Build history of the part. All positions in model axes, mm. A direction names the side the tool comes from. Round coordinates to 2 decimals unless told otherwise and drop trailing zeros. Order: outer loops, then holes, each group sorted by start corner. A loop starts at its lowest first (then second) coordinate and runs counter-clockwise, first axis right, second up. Notation, with made-up numbers: M 20.25,85.25 L 29.25,85.25 A23 ccw 29.25,98.25 Z; hole C 39,87 d6. An arc over 180 degrees is marked long. Use CSV: the item, a comma, the result in double quotes.
from build123d import *

# Parameters (mm, degrees)
BRACKET_BODY_DEPTH           = 12
RECTANGULAR_WINDOW_CUT_DEPTH = 5
KEYHOLE_SLOT_CUT_DEPTH       = 10
EDGE_NOTCH_CUT_DEPTH         = 2


with BuildPart() as part:
    # Bracket Profile Sketch → Bracket Body (new, symmetric)
    with BuildSketch(Plane.XY):
        with BuildLine():
            Line((2, 0), (18.5, 0))
            ThreePointArc((18.5, 0), (19.75, -1.25), (18.5, -2.5))
            Line((18.5, -2.5), (17, -2.5))
            Line((17, -2.5), (17, -1.268700577))
            Line((17, -1.268700577), (18.441553142, -1.268700577))
            ThreePointArc((18.441553142, -1.268700577), (18.497202853, -1.134350288), (18.441553142, -1))
            Line((18.441553142, -1), (3.021384942, -1))
            ThreePointArc((3.021384942, -1), (1.592049942, -1.592049942), (1, -3.021384942))
            Line((1, -3.021384942), (1, -29))
            Line((1, -29), (0, -29))
            Line((0, -29), (0, -2))
            ThreePointArc((0, -2), (0.585786438, -0.585786438), (2, 0))
        make_face()
    extrude(amount=BRACKET_BODY_DEPTH, both=True)

    # Rectangular Window Sketch → Rectangular Window Cut (cut, symmetric)
    with BuildSketch(Plane.XZ.offset(1)):
        with BuildLine():
            Line((8, -6), (14, -6))
            ThreePointArc((14, -6), (15.414213562, -5.414213562), (16, -4))
            Line((16, -4), (16, 4))
            ThreePointArc((16, 4), (15.414213562, 5.414213562), (14, 6))
            Line((14, 6), (8, 6))
            ThreePointArc((8, 6), (6.585786438, 5.414213562), (6, 4))
            Line((6, 4), (6, -4))
            ThreePointArc((6, -4), (6.585786438, -5.414213562), (8, -6))
        make_face()
    extrude(amount=RECTANGULAR_WINDOW_CUT_DEPTH, both=True, mode=Mode.SUBTRACT)

    # Keyhole Slot Sketch → Keyhole Slot Cut (cut)
    with BuildSketch(Plane(origin=(1, 0, 0), x_dir=(0, 0, -1), z_dir=(1, 0, 0))):
        with BuildLine():
            ThreePointArc((7.546363234, -23.655635881), (4.623576141, -27.52859431), (-3.9e-08, -29))
            Line((-3.9e-08, -29), (12, -29))
            Line((12, -29), (12, -11))
            Line((12, -11), (7.546363234, -23.655635881))
        make_face()
        with BuildLine():
            Line((-7.546363234, -23.655635881), (-12, -11))
            Line((-12, -11), (-12, -29))
            Line((-12, -29), (-3.9e-08, -29))
            ThreePointArc((-3.9e-08, -29), (-4.623576172, -27.528594288), (-7.546363234, -23.655635881))
        make_face()
    extrude(amount=-KEYHOLE_SLOT_CUT_DEPTH, mode=Mode.SUBTRACT)

    # Edge Notch Sketch → Edge Notch Cut (cut)
    with BuildSketch(Plane(origin=(1, 0, 0), x_dir=(0, 0, -1), z_dir=(1, 0, 0))):
        with BuildLine():
            Line((-2.38, -15.84), (-2.38, -18.339079107))
            ThreePointArc((-2.38, -18.339079107), (0, -24.57), (2.38, -18.339079107))
            Line((2.38, -18.339079107), (2.38, -15.84))
            ThreePointArc((2.38, -15.84), (0, -13.46), (-2.38, -15.84))
        make_face()
    extrude(amount=-EDGE_NOTCH_CUT_DEPTH, mode=Mode.SUBTRACT)


solid = part.part
(1) Wall check: line 1 (Y direction, x = 18, z = 5.5); line 2 (X direction, y = -9.75, z = 7.75); line 3 (Y direction, x = 6.5, z = 8.5). Give the ranges that are in metal, low to high. Write a range as from..to.
Answer block:
line 1,"y = -2.5..-1.27, -1..0"
line 2,"x = 0..1"
line 3,"y = -1..0"
(2) Two-plate mould, pull along Y, no slides. Class faces 1 (the face through (19.75, -1.22, 0.17)), 2 (the face through (5, 0, 0)), 3 (the face through (18, -1.269, 0)): released by +Y, released by -Y, zero draft, split by the parting line, or undercut.
Answer block:
face 1,"split by the parting line"
face 2,"released by +Y"
face 3,"undercut"
(3) Cut at B-B, the plane y = -21.75. Give the cut face in (x, z).
Answer block:
outline,"M 0,-8.22 L 1,-8.22 L 1,-3.49 L 0,-3.49 Z; M 0,3.49 L 1,3.49 L 1,8.22 L 0,8.22 Z"
(4) Tool access for faces 4 (the face through (0.5, -17.1, -2.38)), 5 (the face through (0.57, -0.6, 0.17)), 6 (the face through (1.608, -1.576, 0.168)), 7 (the face through (6.57, -0.51, -5.4)), 8 (the face through (18, -2.5, 0)): list every direction of +Z, -Z, +X, -X, +Y, -Y with a clear straight run to the whole face (end or side of a thin tool).
Answer block:
face 4,"+X, -X"
face 5,"+Z, -Z, -X, +Y"
face 6,"+Z, -Z, -Y"
face 7,"+Y, -Y"
face 8,"+Z, -Z, +X, -Y"
(5) Cut at D-D, the plane x = 3.5. Give the cut face in (y, z), and give its area (3 significant figures).
Answer block:
outline,"M -1,-12 L 0,-12 L 0,12 L -1,12 Z"
area,"24.0 mm²"
(6) Cut at C-C, the plane z = -5.5. Give the cut face in (x, y).
Answer block:
outline,"M 0,-26.81 L 1,-26.81 L 1,-3.02 A2.02 cw 3.02,-1 L 6.68,-1 L 6.68,0 L 2,0 A2 ccw 0,-2 Z; M 15.32,-1 L 18.44,-1 A0.19 cw 18.44,-1.27 L 17,-1.27 L 17,-2.5 L 18.5,-2.5 A1.25 ccw 18.5,0 L 15.32,0 Z"
(7) Cut at A-A, the plane x = 10.75. Give the cut face in (y, z), and give its area (3 significant figures).
Answer block:
outline,"M -1,-12 L 0,-12 L 0,-6 L -1,-6 Z; M -1,6 L 0,6 L 0,12 L -1,12 Z"
area,"12.0 mm²"
(8) Drop flat-ended pins along their axis: pin 1 (4 mm diameter, centred on y = -25, z = 7.5, fed in from +X); pin 2 (3 mm diameter, centred on x = 3.5, z = 0, fed in from -Y); pin 3 (1.1 mm diameter, centred on y = -0.5, z = 0, fed in from -X). Give the stop position or say it passes through.
Answer block:
pin 1,"stops at x = 1"
pin 2,"stops at y = -1.28"
pin 3,"stops at x = 0.24"
